Input: part model. Units: mm. Frame: model coordinates. A direction names the side the tool comes from. Round coordinates to 2 decimals unless told otherwise and drop trailing zeros. Loops run counter-clockwise (first coordinate to the right, second up) from the corner with the lowest first, then second, coordinate; pieces in that order, holes last. Notation, with made-up numbers: (22.5, 59.5) -> (34.5, 59.5) arc R27 cw to (34.5, 86.5) -> close; hole circle Ø10 at (-22.75, 83). An arc over 180 degrees is marked (long way). Answer in a Markdown table with one row per item. Add a question column.
Q1. Section C-C, the plane y = 84. Output: boundary loops of the cut face in (x, z), and give its area (3 significant figures).
Q2. Section A-A, the plane z = -12.5. Output: boundary loops of the cut face in (x, y).
Q3. Section B-B, the plane x = 35. Output: boundary loops of the cut face in (y, z), and give its area (3 significant figures).
Q4. Section D-D, the plane z = 4.5. Output: boundary loops of the cut face in (x, y), and give its area (3 significant figures).
Q5. Reachability of faces 1 (the face through (1, -6, 0)), 2 (the face through (-32, 97, 18.5)), 3 (the face through (7.5, 101, 37)) from +Z, -Z, +X, -X, +Y, -Y: full face, straight path, thin tool, end or side. Return the list, or none.
Q6. Pin query (flat end, axial travel): pin 1 (2 mm diameter, centred on x = 3, z = -26.5, fed in from +Y); pin 2 (1 mm diameter, centred on x = 55.5, z = 32, fed in from +Y); pin 3 (6 mm diameter, centred on x = 29, z = 38.5, fed in from +Y). Return the tip coordinate at first contact, or that it passes through.
Q7. Ray query, L1, parallel to Y at x = 50, z = 29; L2, parallel to Y at x = 50, z = 35; L3, parallel to Y at x = -20, z = 35. Return the intervals inside material, ascending. Write a range as from..to.
Q8. Mould query, pull axis X, two halves, no side actions, for faces 4 (the face through (14.629, 74.518, 36.584)), 5 (the face through (-42.932, 1.605, -11.459)), 6 (the face through (46, 38, 18.5)), 7 (the face through (56.633, 53.083, 30.668)). Classes: pulls with the +X half, pulls with the -X half, needs draft (parallel to the pull), parting line crosses it, or undercut.
```python
from build123d import *

# Parameters (mm, degrees)
BASE_ANGLE_DEPTH           = 70
PILLAR_WEB_SKETCH_R        = 15
PILLAR_WEB_SKETCH_R_2      = 9
PILLAR_WEB_DEPTH           = 12
BOSS_PROFILES_SKETCH_R     = 9
UPPER_BEARING_BOSS_DEPTH   = 12
LOWER_HUB_BOSS_DEPTH       = 12
LOWER_HUB_BOSS_DEPTH_BACK  = 24
SKETCH5_5_R                = 15
BASE_CUT_REACH             = 157.327
BASE_CUT_SKETCH_R          = 8
BASE_CUT_DIRECTION_2_DEPTH = 156.327074266


with BuildPart() as part:
    # Base Angle Profile Sketch → Base Angle (new, symmetric)
    with BuildSketch(Plane(origin=(0, 0, 0), x_dir=(0, 0, -1), z_dir=(1, 0, 0))):
        Polygon((-24.5, -9), (-24.5, -6), (24.5, -6), (24.5, -9), (42.5, -9), (42.5, 9), (-42.5, 9), (-42.5, -9), align=None)
    extrude(amount=BASE_ANGLE_DEPTH, both=True)

    # Pillar Web Sketch → Pillar Web (add)
    with BuildSketch(Plane(origin=(0, 0, 42.5), x_dir=(-1, 0, 0), z_dir=(0, 0, -1))):
        with BuildLine():
            Line((-70, 47), (-70, 9))
            Line((-70, 9), (70, 9))
            Line((70, 9), (46.866088482, 114.870544241))
            ThreePointArc((46.866088482, 114.870544241), (17.047664759, 136.341062829), (-7.5, 109))
            Line((-7.5, 109), (-7.5, 92))
            ThreePointArc((-7.5, 92), (-14.82233047, 74.32233047), (-32.5, 67))
            Line((-32.5, 67), (-50, 67))
            ThreePointArc((-50, 67), (-64.142135624, 61.142135624), (-70, 47))
        make_face()
        with Locations((20, 109)):
            Circle(PILLAR_WEB_SKETCH_R, mode=Mode.SUBTRACT)
        with Locations((-50, 47)):
            Circle(PILLAR_WEB_SKETCH_R_2, mode=Mode.SUBTRACT)
    extrude(amount=PILLAR_WEB_DEPTH)

    # Boss Profiles Sketch → Upper Bearing Boss (add)
    with BuildSketch(Plane(origin=(0, 0, 30.5), x_dir=(-1, 0, 0), z_dir=(0, 0, -1))):
        with BuildLine():
            ThreePointArc((-70, 47), (-50, 27), (-30, 47))
            ThreePointArc((-30, 47), (-35.857864376, 61.142135624), (-50, 67))
            ThreePointArc((-50, 67), (-64.142135624, 61.142135624), (-70, 47))
        make_face()
        with Locations((-50, 47)):
            Circle(BOSS_PROFILES_SKETCH_R, mode=Mode.SUBTRACT)
    extrude(amount=UPPER_BEARING_BOSS_DEPTH)

    # Sketch5_5 → Lower Hub Boss (add, two sides: drawn at the far end of the back side and taken through both)
    with BuildSketch(Plane(origin=(0, 0, 30.5), x_dir=(-1, 0, 0), z_dir=(0, 0, -1)).offset(-LOWER_HUB_BOSS_DEPTH_BACK)):
        with BuildLine():
            ThreePointArc((-7.5, 109), (20, 81.5), (47.5, 109))
            ThreePointArc((47.5, 109), (47.341062829, 111.952335241), (46.866088482, 114.870544241))
            ThreePointArc((46.866088482, 114.870544241), (17.047664759, 136.341062829), (-7.5, 109))
        make_face()
        with Locations((20, 109)):
            Circle(SKETCH5_5_R, mode=Mode.SUBTRACT)
    extrude(amount=LOWER_HUB_BOSS_DEPTH + LOWER_HUB_BOSS_DEPTH_BACK)

    # Base Cut Sketch → Base Cut (cut, up to next)
    with BuildSketch(Plane(origin=(0, 9, 0), x_dir=(1, 0, 0), z_dir=(0, 1, 0)), mode=Mode.PRIVATE) as base_cut_sk1:
        with Locations(Location((-35, 12.5, 0), (0, 0, 90))):
            Circle(BASE_CUT_SKETCH_R)
    base_cut_tool1 = extrude(base_cut_sk1.sketch, amount=-BASE_CUT_REACH, mode=Mode.PRIVATE) & part.part
    # Base Cut Sketch → Base Cut (cut, up to next)
    with BuildSketch(Plane(origin=(0, 9, 0), x_dir=(1, 0, 0), z_dir=(0, 1, 0)), mode=Mode.PRIVATE) as base_cut_sk2:
        with Locations(Location((35, 12.5, 0), (0, 0, 90))):
            Circle(BASE_CUT_SKETCH_R)
    base_cut_tool2 = extrude(base_cut_sk2.sketch, amount=-BASE_CUT_REACH, mode=Mode.PRIVATE) & part.part
    add(base_cut_tool1.solids().sort_by_distance((-35, 9, -12.5))[0], mode=Mode.SUBTRACT)
    add(base_cut_tool2.solids().sort_by_distance((35, 9, -12.5))[0], mode=Mode.SUBTRACT)

    # Base Cut Sketch → Base Cut direction 2 (cut)
    with BuildSketch(Plane(origin=(0, 9, 0), x_dir=(1, 0, 0), z_dir=(0, 1, 0))):
        with Locations(Location((-35, 12.5, 0), (0, 0, 90))):
            Circle(BASE_CUT_SKETCH_R)
        with Locations(Location((35, 12.5, 0), (0, 0, 90))):
            Circle(BASE_CUT_SKETCH_R)
    extrude(amount=BASE_CUT_DIRECTION_2_DEPTH, mode=Mode.SUBTRACT)


solid = part.part
```
Answer block:
| question | item | result |
|---|---|---|
| 1 | outline | (-53.61, 30.5) -> (-31.46, 30.5) -> (-31.46, 18.5) -> (-8.54, 18.5) -> (-8.54, 30.5) -> (8.81, 30.5) -> (8.81, 42.5) -> (-8.54, 42.5) -> (-8.54, 54.5) -> (-31.46, 54.5) -> (-31.46, 42.5) -> (-53.61, 42.5) -> close |
| 1 | area | 1,300 mm^2 |
| 2 | outline | (-70, -6) -> (-43, -6) -> (-43, 9) -> (-70, 9) -> close; (-27, -6) -> (27, -6) -> (27, 9) -> (-27, 9) -> close; (43, -6) -> (70, -6) -> (70, 9) -> (43, 9) -> close |
| 3 | outline | (-9, -42.5) -> (9, -42.5) -> (9, -20.5) -> (-6, -20.5) -> (-6, -24.5) -> (-9, -24.5) -> close; (-9, 24.5) -> (-6, 24.5) -> (-6, -4.5) -> (9, -4.5) -> (9, 30.5) -> (33.77, 30.5) -> (33.77, 18.5) -> (60.23, 18.5) -> (60.23, 30.5) -> (67, 30.5) -> (67, 42.5) -> (-9, 42.5) -> close |
| 3 | area | 2,160 mm^2 |
| 4 | outline | (-70, -6) -> (70, -6) -> (70, 9) -> (-70, 9) -> close |
| 4 | area | 2,100 mm^2 |
| 5 | face 1 | +X, -X, -Y |
| 5 | face 2 | -Z, +X, -X, +Y |
| 5 | face 3 | +Z, -Z, +X, +Y |
| 6 | pin 1 | y = 9 |
| 6 | pin 2 | y = 66.36 |
| 6 | pin 3 | y = 67.86 |
| 7 | L1 | -9..9, 27..38, 56..67 |
| 7 | L2 | -9..38, 56..67 |
| 7 | L3 | -9..94, 124..136.5 |
| 8 | face 4 | pulls with the +X half |
| 8 | face 5 | undercut |
| 8 | face 6 | needs draft |
| 8 | face 7 | undercut |
